The model under review builds one solid part; all positions refer to its coordinate system, in mm. A direction names the side the tool comes from. Round coordinates to 2 decimals unless told otherwise and drop trailing zeros. Order: outer loops, then holes, each group sorted by start corner. A loop starts at its lowest first (then second) coordinate and runs counter-clockwise, first axis right, second up. Notation, with made-up numbers: (-27, 24.5) -> (14, 24.5) arc R10 ccw to (14, 32.5) -> close; hole circle Ø6 at (-17.5, 20.5). An arc over 180 degrees is marked (long way). Put each result on its own line as item: value. Start each with the question number.
from build123d import *

# Parameters (mm, degrees)
SKETCH_1_3_W        = 20
SKETCH_1_3_H        = 80
BOSS_EXTRUDE1_DEPTH = 8.5
SKETCH_1_3_2_W      = 24.5
SKETCH_1_3_2_H      = 80
SKETCH_1_3_2_R      = 5.5
BOSS_EXTRUDE2_DEPTH = 20


with BuildPart() as part:
    # Sketch 1_3 → Boss-Extrude1 (new body)
    with BuildSketch(Plane(origin=(0, 0, 0), x_dir=(0, 0, -1), z_dir=(1, 0, 0))):
        with Locations((-12.25, 0)):
            Rectangle(SKETCH_1_3_W, SKETCH_1_3_H)
    extrude(amount=BOSS_EXTRUDE1_DEPTH)

    # Sketch 1_3 2 → Boss-Extrude2 (add)
    with BuildSketch(Plane(origin=(0, 0, 0), x_dir=(0, 0, -1), z_dir=(1, 0, 0))):
        with Locations((10, 0)):
            Rectangle(SKETCH_1_3_2_W, SKETCH_1_3_2_H)
        with Locations((12.25, -20)):
            Circle(SKETCH_1_3_2_R, mode=Mode.SUBTRACT)
        with Locations((12.25, 20)):
            Circle(SKETCH_1_3_2_R, mode=Mode.SUBTRACT)
    extrude(amount=BOSS_EXTRUDE2_DEPTH)


solid = part.part
Q1. Draft analysis for pull direction Z (two halves, no side actions). For faces 3 (the face through (9.86, -22.11, -17.33)), 4 (the face through (20, 1, -10)), 5 (the face through (9.86, 24.638, -15.207)), 6 (the face through (10, -1, -22.25)), state which applies: +Z half, -Z half, draft (parallel to the pull), parting line (faces both ways), or undercut.
Q2. Take a section at C-C on y = 20. Give the boundary of the cut face in (x, z), and give its area (3 significant figures).
Q3. Take a section at B-B on x = 12.5. Give the boundary of the cut face in (y, z).
Q4. For faces 1 (the face through (14, -1, 2.25)), 2 (the face through (0, 1, 0)), list the 3-axis set-ups (+Z, -Z, +X, -X, +Y, -Y) from which the entire face can be reached by the end or side of a thin tool; tool diameter is ignored.
Q5. Wall thickness on probe 1 along Y at (x, z) = (1.25, -12.5); probe 2 along Y at (x, z) = (11.5, -11); probe 3 along Z at (x, y) = (7.25, 15): over which ranges is each line inside the solid? List them lowest first. Write a range as [from, to].
Q6. Clearance check with flat-ended pins moving along their axes: pin 1 Ø10 at (y, z) = (-3.5, 13) entering from +X; pin 2 Ø2 at (x, y) = (12, 27.5) entering from +Z. State where each tip first meets the part, or that it passes through.
Q7. Take a section at D-D on z = 15. Give the boundary of the cut face in (x, y), and give its area (3 significant figures).
Q8. Take a section at A-A on z = -12.25. Give the boundary of the cut face in (x, y), and give its area (3 significant figures).
Calculated:
1. face 3: undercut
1. face 4: draft
1. face 5: undercut
1. face 6: -Z half
2. outline: (0, -22.25) -> (20, -22.25) -> (20, -17.75) -> (0, -17.75) -> close; (0, -6.75) -> (20, -6.75) -> (20, 2.25) -> (8.5, 2.25) -> (8.5, 22.25) -> (0, 22.25) -> close
2. area: 440 mm²
3. outline: (-40, -22.25) -> (40, -22.25) -> (40, 2.25) -> (-40, 2.25) -> close; hole circle Ø11 at (-20, -12.25); hole circle Ø11 at (20, -12.25)
4. face 1: +Z, +X, +Y, -Y
4. face 2: +Z, -Z, -X, +Y, -Y
5. probe 1: y = [-40, -25.49], [-14.51, 14.51], [25.49, 40]
5. probe 2: y = [-40, -25.36], [-14.64, 14.64], [25.36, 40]
5. probe 3: z = [-22.25, -14.54], [-9.96, 22.25]
6. pin 1: stops at x = 8.5
6. pin 2: stops at z = 2.25
7. outline: (0, -40) -> (8.5, -40) -> (8.5, 40) -> (0, 40) -> close
7. area: 680 mm²
8. outline: (0, -40) -> (20, -40) -> (20, -25.5) -> (0, -25.5) -> close; (0, -14.5) -> (20, -14.5) -> (20, 14.5) -> (0, 14.5) -> close; (0, 25.5) -> (20, 25.5) -> (20, 40) -> (0, 40) -> close
8. area: 1,160 mm²
